Verification items for the finished model (mm, model axes). A direction names the side the tool comes from. Give positions to 0.01 mm unless a question says otherwise; leave off trailing zeros. Loops run counter-clockwise (first coordinate to the right, second up) from the corner with the lowest first, then second, coordinate; pieces in that order, holes last. Notation, with made-up numbers: (49.25, 42) -> (84.25, 42) arc R15 ccw to (84.25, 61) -> close; hole circle Ø2 at (71.25, 13). An arc over 180 degrees is marked (long way). Use one line per item in the form item = value. Start each with the question number.
from build123d import *

# Parameters (mm, degrees)
BOSS_EXTRUDE2_DEPTH       = 325
BOSS_EXTRUDE2_2_DEPTH     = 325
BOSS_EXTRUDE3_DEPTH       = 4
BOSS_EXTRUDE4_START       = -4
BOSS_EXTRUDE4_DEPTH       = 4
SKETCH5_R                 = 6
CUT_EXTRUDE1_DEPTH        = 10
LPATTERN1_COUNT           = 3
LPATTERN1_PITCH           = 150
LPATTERN2_COPY_1_SKETCH_R = 6
LPATTERN2_COPY_1_DEPTH    = 10
LPATTERN2_COPY_2_SKETCH_R = 6
LPATTERN2_COPY_2_DEPTH    = 10
LPATTERN2_COPY_3_SKETCH_R = 6
LPATTERN2_COPY_3_DEPTH    = 10
LPATTERN2_COPY_4_SKETCH_R = 6
LPATTERN2_COPY_4_DEPTH    = 10
LPATTERN2_COPY_5_SKETCH_R = 6
LPATTERN2_COPY_5_DEPTH    = 10
LPATTERN2_COPY_6_SKETCH_R = 6
LPATTERN2_COPY_6_DEPTH    = 10
CUT_EXTRUDE2_DEPTH        = 762.052386329
CUT_EXTRUDE2_DEPTH_BACK   = 762.052386329
SKETCH6_R                 = 17.5
CUT_EXTRUDE3_DEPTH        = 762.052386329
CUT_EXTRUDE3_DEPTH_BACK   = 762.052386329
SKETCH7_W                 = 100.370226039
SKETCH7_H                 = 50
SKETCH8_W                 = 650
SKETCH8_H                 = 8
BOSS_EXTRUDE5_DEPTH       = 42.141012962
CUT_EXTRUDE4_DEPTH        = 762.052386329
CUT_EXTRUDE4_DEPTH_BACK   = 762.052386329
SKETCH9_W                 = 99.024260435
SKETCH9_H                 = 85.798945111
SKETCH10_W                = 50
SKETCH10_H                = 54
BOSS_EXTRUDE6_DEPTH       = 8


with BuildPart() as part:
    # Sketch1 → Boss-Extrude2 (new, symmetric)
    with BuildSketch(Plane.XY):
        with BuildLine():
            Line((-223, 0), (-277, 0))
            Line((-277, 0), (-277, -8))
            Line((-277, -8), (-234.858987038, -8))
            Line((-234.858987038, -8), (-234.858987038, -219.476006061))
            Line((-234.858987038, -219.476006061), (-278.858987038, -219.476006061))
            Line((-278.858987038, -219.476006061), (-278.858987038, -227.476006061))
            Line((-278.858987038, -227.476006061), (-226.858987038, -227.476006061))
            Line((-226.858987038, -227.476006061), (-226.858987038, -8))
            ThreePointArc((-226.858987038, -8), (-194.556923413, -116.947011728), (-113.5, -196.587766659))
            Line((-113.5, -196.587766659), (-60, -227.476006061))
            Line((-60, -227.476006061), (-58, -224.011904446))
            Line((-58, -224.011904446), (-111.5, -193.123665044))
            ThreePointArc((-111.5, -193.123665044), (-193.123665044, -111.5), (-223, 0))
        make_face()
    extrude(amount=BOSS_EXTRUDE2_DEPTH, both=True)



with BuildPart() as body_2:
    # Sketch1 → Boss-Extrude2 2 (new, symmetric)
    with BuildSketch(Plane.XY):
        Polygon((277, 0), (223, 0), (223, -177.199169847), (-51.368080573, -277.060984409), (-50, -280.819754892), (227, -180), (227, -227.476006061), (279, -227.476006061), (279, -219.476006061), (235, -219.476006061), (235, -8), (277, -8), align=None)
    extrude(amount=BOSS_EXTRUDE2_2_DEPTH, both=True)


with BuildPart() as part_1:
    add(part.part)

    add(body_2.part)  # Boss-Extrude3 merges body 2
    # Sketch3 → Boss-Extrude3 (add)
    with BuildSketch(Plane.XY.offset(325)):
        with BuildLine():
            Line((-58, -224.011904446), (-60, -227.476006061))
            Line((-60, -227.476006061), (84.865527782, -227.476006061))
            Line((84.865527782, -227.476006061), (223, -177.199169847))
            Line((223, -177.199169847), (223, 0))
            Line((223, 0), (-223, 0))
            ThreePointArc((-223, 0), (-193.123665044, -111.5), (-111.5, -193.123665044))
            Line((-111.5, -193.123665044), (-58, -224.011904446))
        make_face()
        Polygon((84.865527782, -227.476006061), (-60, -227.476006061), (-50.747008298, -276.834932587), align=None)
    extrude(amount=-BOSS_EXTRUDE3_DEPTH)

    # Sketch4 → Boss-Extrude4 (add)
    with BuildSketch(Plane(origin=(0, 0, -325), x_dir=(-1, 0, 0), z_dir=(0, 0, -1)).offset(BOSS_EXTRUDE4_START)):
        with BuildLine():
            Line((111.5, -193.123665044), (58, -224.011904446))
            Line((58, -224.011904446), (60, -227.476006061))
            Line((60, -227.476006061), (51.368080573, -277.060984409))
            Line((51.368080573, -277.060984409), (-223, -177.199169847))
            Line((-223, -177.199169847), (-223, 0))
            Line((-223, 0), (223, 0))
            ThreePointArc((223, 0), (193.123665044, -111.5), (111.5, -193.123665044))
        make_face()
    extrude(amount=BOSS_EXTRUDE4_DEPTH)

    # Sketch5 → Cut-Extrude1 (cut)
    with BuildSketch(Plane(origin=(0, 0, 0), x_dir=(1, 0, 0), z_dir=(0, 1, 0))):
        with Locations(Location((-257, 0, 0), (0, 0, 180))):
            Circle(SKETCH5_R)
        with Locations(Location((259, 0, 0), (0, 0, 180))):
            Circle(SKETCH5_R)
    cut_extrude1 = extrude(amount=-CUT_EXTRUDE1_DEPTH, mode=Mode.SUBTRACT)

    # LPattern1: Cut-Extrude1 ×3
    with Locations(*[(0, 0, -i * LPATTERN1_PITCH) for i in range(1, LPATTERN1_COUNT)]):
        add(cut_extrude1, mode=Mode.SUBTRACT)

    # LPattern2 copy 1 sketch → LPattern2 copy 1 (cut)
    with BuildSketch(Plane(origin=(0, 0, 0), x_dir=(1, 0, 0), z_dir=(0, 1, 0))):
        with Locations(Location((-257, 0, 0), (0, 0, 180))):
            Circle(LPATTERN2_COPY_1_SKETCH_R)
        with Locations(Location((259, 0, 0), (0, 0, 180))):
            Circle(LPATTERN2_COPY_1_SKETCH_R)
    extrude(amount=-LPATTERN2_COPY_1_DEPTH, mode=Mode.SUBTRACT)

    # LPattern2 copy 2 sketch → LPattern2 copy 2 (cut)
    with BuildSketch(Plane(origin=(0, 0, 150), x_dir=(1, 0, 0), z_dir=(0, 1, 0))):
        with Locations(Location((-257, 0, 0), (0, 0, 180))):
            Circle(LPATTERN2_COPY_2_SKETCH_R)
        with Locations(Location((259, 0, 0), (0, 0, 180))):
            Circle(LPATTERN2_COPY_2_SKETCH_R)
    extrude(amount=-LPATTERN2_COPY_2_DEPTH, mode=Mode.SUBTRACT)

    # LPattern2 copy 3 sketch → LPattern2 copy 3 (cut)
    with BuildSketch(Plane(origin=(0, 0, -150), x_dir=(1, 0, 0), z_dir=(0, 1, 0))):
        with Locations(Location((-257, 0, 0), (0, 0, 180))):
            Circle(LPATTERN2_COPY_3_SKETCH_R)
        with Locations(Location((259, 0, 0), (0, 0, 180))):
            Circle(LPATTERN2_COPY_3_SKETCH_R)
    extrude(amount=-LPATTERN2_COPY_3_DEPTH, mode=Mode.SUBTRACT)

    # LPattern2 copy 4 sketch → LPattern2 copy 4 (cut)
    with BuildSketch(Plane(origin=(0, 0, 0), x_dir=(1, 0, 0), z_dir=(0, 1, 0))):
        with Locations(Location((-257, 0, 0), (0, 0, 180))):
            Circle(LPATTERN2_COPY_4_SKETCH_R)
        with Locations(Location((259, 0, 0), (0, 0, 180))):
            Circle(LPATTERN2_COPY_4_SKETCH_R)
    extrude(amount=-LPATTERN2_COPY_4_DEPTH, mode=Mode.SUBTRACT)

    # LPattern2 copy 5 sketch → LPattern2 copy 5 (cut)
    with BuildSketch(Plane(origin=(0, 0, 150), x_dir=(1, 0, 0), z_dir=(0, 1, 0))):
        with Locations(Location((-257, 0, 0), (0, 0, 180))):
            Circle(LPATTERN2_COPY_5_SKETCH_R)
        with Locations(Location((259, 0, 0), (0, 0, 180))):
            Circle(LPATTERN2_COPY_5_SKETCH_R)
    extrude(amount=-LPATTERN2_COPY_5_DEPTH, mode=Mode.SUBTRACT)

    # LPattern2 copy 6 sketch → LPattern2 copy 6 (cut)
    with BuildSketch(Plane(origin=(0, 0, 300), x_dir=(1, 0, 0), z_dir=(0, 1, 0))):
        with Locations(Location((-257, 0, 0), (0, 0, 180))):
            Circle(LPATTERN2_COPY_6_SKETCH_R)
        with Locations(Location((259, 0, 0), (0, 0, 180))):
            Circle(LPATTERN2_COPY_6_SKETCH_R)
    extrude(amount=-LPATTERN2_COPY_6_DEPTH, mode=Mode.SUBTRACT)

    # Sketch6 → Cut-Extrude2 (cut, two sides: drawn at the far end of the back side and taken through both)
    with BuildSketch(Plane(origin=(0, 0, -325), x_dir=(-1, 0, 0), z_dir=(0, 0, -1)).offset(-CUT_EXTRUDE2_DEPTH_BACK)):
        Circle(SKETCH6_R)
    extrude(amount=CUT_EXTRUDE2_DEPTH + CUT_EXTRUDE2_DEPTH_BACK, mode=Mode.SUBTRACT)

    # Sketch7 → Cut-Extrude3 (cut, two sides: drawn at the far end of the back side and taken through both)
    with BuildSketch(Plane.XY.offset(325).offset(-CUT_EXTRUDE3_DEPTH_BACK)):
        with Locations((-277.044100058, -202.476006061)):
            Rectangle(SKETCH7_W, SKETCH7_H)
    extrude(amount=CUT_EXTRUDE3_DEPTH + CUT_EXTRUDE3_DEPTH_BACK, mode=Mode.SUBTRACT)

    # Sketch8 → Boss-Extrude5 (add)
    with BuildSketch(Plane.ZY.offset(234.858987038)):
        with Locations((0, -173.476006061)):
            Rectangle(SKETCH8_W, SKETCH8_H)
    extrude(amount=BOSS_EXTRUDE5_DEPTH)

    # Sketch9 → Cut-Extrude4 (cut, two sides: drawn at the far end of the back side and taken through both)
    with BuildSketch(Plane.XY.offset(325).offset(-CUT_EXTRUDE4_DEPTH_BACK)):
        with Locations((276.512130218, -222.899472556)):
            Rectangle(SKETCH9_W, SKETCH9_H)
    extrude(amount=CUT_EXTRUDE4_DEPTH + CUT_EXTRUDE4_DEPTH_BACK, mode=Mode.SUBTRACT)

    # Sketch10 → Boss-Extrude6 (add)
    with BuildSketch(Plane(origin=(0, 0, 0), x_dir=(1, 0, 0), z_dir=(0, 1, 0))):
        with Locations((-252, 352)):
            Rectangle(SKETCH10_W, SKETCH10_H)
        with Locations((252, 352)):
            Rectangle(SKETCH10_W, SKETCH10_H)
        with Locations((252, -352)):
            Rectangle(SKETCH10_W, SKETCH10_H)
        with Locations((-252, -352)):
            Rectangle(SKETCH10_W, SKETCH10_H)
    extrude(amount=-BOSS_EXTRUDE6_DEPTH)


solid = part_1.part
Item 1: Material ranges on line 1 (X direction, y = -5, z = -300); line 2 (Z direction, x = 259, y = -5.25); line 3 (X direction, y = -2.5, z = -300), recorded low to high.
Item 2: Sectioned sample at A-A, the plane y = -95.5. Enter the section's corners in (x, z), and give its area (3 significant figures).
Item 3: Sectioned sample at C-C, the plane x = -162.5. Enter the section's corners in (y, z).
Item 4: Gauge pin test, flat ends, axial feed: pin 1 Ø4 at (x, z) = (39, -161.5) entering from +Y; pin 2 Ø10 at (x, y) = (-128, -98) entering from +Z; pin 3 Ø6 at (x, z) = (-90, 85) entering from +Y; pin 4 Ø9.5 at (x, z) = (259, 150) entering from +Y. Record the tip position at first contact, or that the pin passes through.
Item 5: Sectioned sample at B-B, the plane z = 42. Enter the section's corners in (x, y), and give its area (3 significant figures).
Item 6: Tool access check on faces 1 (the cylindrical face through (0.385, -17.496, -322.972)), 2 (the flat face through (-252, -177.476, -5)), 3 (the cylindrical face through (-192.301, -112.913, 4.494)), 4 (the flat face through (-256, -169.476, -5)), 5 (the flat face through (244, 0, 2)). Record the directions out of +Z, -Z, +X, -X, +Y, -Y that give a thin tool (end or side, any length) a straight path to the whole face; none if there is none.
Item 7: Draft check along Y on faces 6 (the flat face through (-252, -8, -5)), 7 (the flat face through (-234.859, -88, 5)), 8 (the flat face through (235, -95, 5)), 9 (the flat face through (87.74, -226.43, 6.52)). Enter one of: +Y half, -Y half, draft (parallel to the pull), parting line (faces both ways), or undercut.
Item 8: Sectioned sample at D-D, the plane x = 44.5. Enter the section's corners in (y, z), and give its area (3 significant figures).
Outcome:
q1.line_1 = -277 to -263, -251 to -222.94, 223 to 253, 265 to 277
q1.line_2 = -379 to -306, -294 to -156, -144 to -6, 6 to 144, 156 to 294, 306 to 379
q1.line_3 = -277 to -263, -251 to -222.99, 223 to 253, 265 to 277
q2.outline = (-234.86, -325) -> (-226.86, -325) -> (-226.86, 325) -> (-234.86, 325) -> close; (-205.93, -325) -> (235, -325) -> (235, 325) -> (-205.93, 325) -> close; hole (-201.52, -321) -> (223, -321) -> (223, 321) -> (-201.52, 321) -> close
q2.area = 19,300 mm^2
q3.outline = (-158.5, -325) -> (0, -325) -> (0, -321) -> (-152.72, -321) -> (-152.72, 321) -> (0, 321) -> (0, 325) -> (-158.5, 325) -> close
q4.pin_1 = -243.44
q4.pin_2 = 325
q4.pin_3 = -203.8
q4.pin_4 = through
q5.outline = (-277, -177.48) -> (-226.86, -177.48) -> (-226.86, -8) arc R227 ccw to (-113.5, -196.59) -> (-60, -227.48) -> (-58, -224.01) -> (-111.5, -193.12) arc R223 cw to (-223, 0) -> (-277, 0) -> (-277, -8) -> (-234.86, -8) -> (-234.86, -169.48) -> (-277, -169.48) -> close; (-51.37, -277.06) -> (-50, -280.82) -> (227, -180) -> (235, -180) -> (235, -8) -> (277, -8) -> (277, 0) -> (223, 0) -> (223, -177.2) -> close
q5.area = 6,950 mm^2
q6.face_1 = +Z, -Z, +Y
q6.face_2 = +Z, -Z, -X, -Y
q6.face_3 = +Y
q6.face_4 = +Z, -Z, -X
q6.face_5 = +Z, -Z, +X, -X, +Y
q7.face_6 = undercut
q7.face_7 = undercut
q7.face_8 = draft
q7.face_9 = +Y half
q8.outline = (-246.42, -325) -> (0, -325) -> (0, -321) -> (-242.17, -321) -> (-242.17, 321) -> (0, 321) -> (0, 325) -> (-246.42, 325) -> close
q8.area = 4,700 mm^2
